Geometry check sheet. Reference: the model listing, model coordinates, mm. Round coordinates to 2 decimals unless told otherwise and drop trailing zeros. Order: outer loops, then holes, each group sorted by start corner. A loop starts at its lowest first (then second) coordinate and runs counter-clockwise, first axis right, second up. Notation, with made-up numbers: (13.25, 82) -> (24.25, 82) arc R13 ccw to (24.25, 91) -> close; hole circle Ø7 at (76, 30.5). An arc over 180 degrees is marked (long way). Use a Markdown table: item, result. Add a question column.
Item 1: Material ranges on probe 1 along Y at (x, z) = (433.5, 10.5); probe 2 along Y at (x, z) = (358.5, 2.5); probe 3 along X at (y, z) = (65.5, 7.75), recorded low to high. Write a range as [from, to].
Item 2: Sectioned sample at B-B, the plane x = 340. Record the cut outline in (y, z), and give its area (3 significant figures).
Item 3: Sectioned sample at A-A, the plane z = 10. Record the cut outline in (x, y), and give its area (3 significant figures).
Item 4: Gauge pin test, flat ends, axial feed: pin 1 Ø8.5 at (x, y) = (270, 93) entering from +Z; pin 2 Ø3.5 at (x, y) = (189.5, 9) entering from -Z; pin 3 Ø7.5 at (x, y) = (103.5, 10.55) entering from +Z. Record the tip position at first contact, or that the pin passes through.
from build123d import *

# Parameters (mm, degrees)
SKETCH_1_W                   = 462
SKETCH_1_H                   = 100
EXTRUDE_1_DEPTH              = 12
SKETCH_2_W                   = 462
SKETCH_2_H                   = 15.1
CUT_EXTRUDE_1_DEPTH          = 4
HOLE_WIZARD_M6_1_D           = 6.6
HOLE_WIZARD_M6_1_CBORE_D     = 11
HOLE_WIZARD_M6_1_CBORE_DEPTH = 6.4
SKETCH_5_R                   = 10
CUT_EXTRUDE_2_DEPTH          = 2
HOLE_WIZARD_M6_2_D           = 6.6
HOLE_WIZARD_M6_2_CBORE_D     = 11
HOLE_WIZARD_M6_2_CBORE_DEPTH = 6.4
HOLE_WIZARD_M6_3_D           = 6.6
HOLE_WIZARD_M6_3_CBORE_D     = 11
HOLE_WIZARD_M6_3_CBORE_DEPTH = 6.4
CHAMFER_1_SIZE               = 5


with BuildPart() as part:
    # 草图1 → 凸台-拉伸1 (new body)
    with BuildSketch(Plane.XY):
        with Locations((231, 50)):
            Rectangle(SKETCH_1_W, SKETCH_1_H)
    extrude(amount=EXTRUDE_1_DEPTH)

    # 草图2 → 切除-拉伸1 (cut)
    with BuildSketch(Plane.XY.offset(12)):
        with Locations((231, 10.55)):
            Rectangle(SKETCH_2_W, SKETCH_2_H)
    extrude(amount=-CUT_EXTRUDE_1_DEPTH, mode=Mode.SUBTRACT)

    # M6 六角凹头螺钉的柱形沉头孔1 (through all)
    with Locations(Plane.XY.offset(12)):
        with Locations((192, 93), (270, 93), (192, 67), (270, 67)):
            CounterBoreHole(HOLE_WIZARD_M6_1_D / 2, HOLE_WIZARD_M6_1_CBORE_D / 2, HOLE_WIZARD_M6_1_CBORE_DEPTH)

    # 草图5 → 切除-拉伸2 (cut)
    with BuildSketch(Plane(origin=(0, 0, 0), x_dir=(-1, 0, 0), z_dir=(0, 0, -1))):
        with Locations((-387, 80)):
            Circle(SKETCH_5_R)
        with Locations((-75, 80)):
            Circle(SKETCH_5_R)
    extrude(amount=-CUT_EXTRUDE_2_DEPTH, mode=Mode.SUBTRACT)

    # M6 六角凹头螺钉的柱形沉头孔2 (through all)
    with Locations(Plane.XY.offset(12)):
        with Locations((75, 80), (387, 80)):
            CounterBoreHole(HOLE_WIZARD_M6_2_D / 2, HOLE_WIZARD_M6_2_CBORE_D / 2, HOLE_WIZARD_M6_2_CBORE_DEPTH)

    # M6 六角凹头螺钉的柱形沉头孔3 (through all)
    with Locations(Plane(origin=(0, 0, 0), x_dir=(-1, 0, 0), z_dir=(0, 0, -1))):
        with Locations((-443.5, 10.55), (-358.5, 10.55), (-273.5, 10.55), (-188.5, 10.55), (-103.5, 10.55), (-18.5, 10.55)):
            CounterBoreHole(HOLE_WIZARD_M6_3_D / 2, HOLE_WIZARD_M6_3_CBORE_D / 2, HOLE_WIZARD_M6_3_CBORE_DEPTH)

    # 倒角1
    chamfer_1_edges = [part.edges().sort_by_distance(p)[0] for p in [
        (0, 100, 6),
        (462, 100, 6),
    ]]
    chamfer(chamfer_1_edges, length=CHAMFER_1_SIZE)


solid = part.part
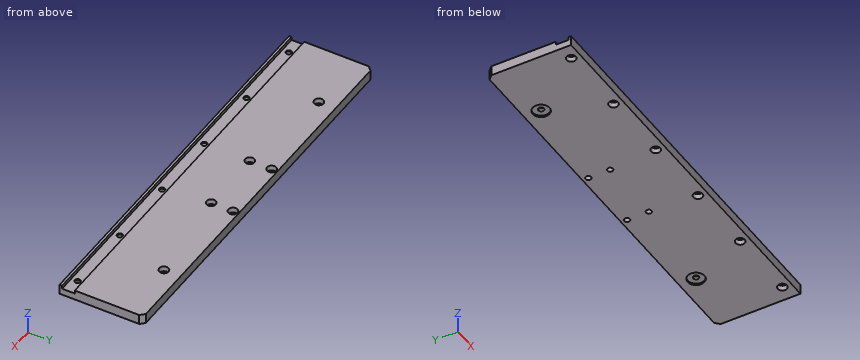
Found:
| question | item | result |
|---|---|---|
| 1 | probe 1 | y = [0, 3], [18.1, 100] |
| 1 | probe 2 | y = [0, 5.05], [16.05, 100] |
| 1 | probe 3 | x = [0, 186.71], [197.29, 264.71], [275.29, 462] |
| 2 | outline | (0, 0) -> (100, 0) -> (100, 12) -> (18.1, 12) -> (18.1, 8) -> (3, 8) -> (3, 12) -> (0, 12) -> close |
| 2 | area | 1,140 mm2 |
| 3 | outline | (0, 0) -> (462, 0) -> (462, 3) -> (0, 3) -> close; (0, 18.1) -> (462, 18.1) -> (462, 95) -> (457, 100) -> (5, 100) -> (0, 95) -> close; hole circle Ø11 at (75, 80); hole circle Ø11 at (192, 67); hole circle Ø11 at (192, 93); hole circle Ø11 at (270, 67); hole circle Ø11 at (270, 93); hole circle Ø11 at (387, 80) |
| 3 | area | 38,600 mm2 |
| 4 | pin 1 | stops at z = 5.6 |
| 4 | pin 2 | stops at z = 6.4 |
| 4 | pin 3 | stops at z = 8 |
